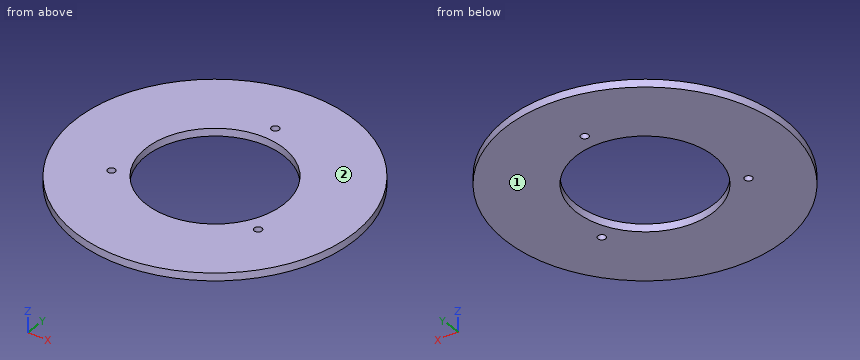
```python
from build123d import *

# Parameters (mm, degrees)
SKETCH1_R           = 91
SKETCH1_R_2         = 45
SKETCH1_R_3         = 2.5
BOSS_EXTRUDE1_DEPTH = 5


with BuildPart() as part:
    # Sketch1 → Boss-Extrude1 (new body)
    with BuildSketch(Plane.XY):
        Circle(SKETCH1_R)
        Circle(SKETCH1_R_2, mode=Mode.SUBTRACT)
        with Locations((0, 55)):
            Circle(SKETCH1_R_3, mode=Mode.SUBTRACT)
        with Locations((47.631397208, -27.5)):
            Circle(SKETCH1_R_3, mode=Mode.SUBTRACT)
        with Locations((-47.631397208, -27.5)):
            Circle(SKETCH1_R_3, mode=Mode.SUBTRACT)
    extrude(amount=BOSS_EXTRUDE1_DEPTH)


solid = part.part
```
For this review, take the finished solid that the model builds, in its own axes (mm). Face numbers are marked on the shaded views. Coordinates: 2 decimals unless noted, no trailing zeros. Loops run counter-clockwise (first coordinate to the right, second up) from the corner with the lowest first, then second, coordinate; pieces in that order, holes last. Notation, with made-up numbers: (73, 85.25) - (85, 85.25) arc R20 ccw to (85, 112.25) - close; hole circle Ø5 at (76, 28.25). An arc over 180 degrees is marked (long way). Use one line per item in the form item = value. Start each with the question number.
1) To check wall thickness, follow probe 1 along Y at (x, z) = (0, 1.85); probe 2 along X at (y, z) = (9, 0.35); probe 3 along X at (y, z) = (36, 3.05). State the ranges of each line that lie inside material, in increasing order. Write a range as from..to.
2) Take a section at D-D (y = -27.5). State the section outline as (x, z) points, plus the area to 3 significant figures.
3) Take a section at A-A (x = 0). State the section outline as (y, z) points.
4) Take a section at C-C (z = 2.8). State the section outline as (x, y) points.
5) For pin 1 (1 mm diameter, centred on x = -13, z = 2, fed in from -Y); pin 2 (3 mm diameter, centred on x = 0, y = 55, fed in from -Z); pin 3 (1 mm diameter, centred on y = 58.5, z = 0.5, fed in from -X); pin 4 (1.5 mm diameter, centred on x = -37, z = 2, fed in from +Y), all flat-tipped, find the tip position at first contact; note any pin that passes through.
6) Take a section at B-B (y = 0). State the section outline as (x, z) points.
7) Draft analysis for pull direction Z (two halves, no side actions). For the marked faces 1 and 2, state which applies: released by +Z, released by -Z, zero draft, split by the parting line, or undercut.
From the geometry:
q1.probe_1 = -91..-45, 45..52.5, 57.5..91
q1.probe_2 = -90.55..-44.09, 44.09..90.55
q1.probe_3 = -83.58..-27, 27..83.58
q2.outline = (-86.75, 0) - (-50.13, 0) - (-50.13, 5) - (-86.75, 5) - close; (-45.13, 0) - (-35.62, 0) - (-35.62, 5) - (-45.13, 5) - close; (35.62, 0) - (45.13, 0) - (45.13, 5) - (35.62, 5) - close; (50.13, 0) - (86.75, 0) - (86.75, 5) - (50.13, 5) - close
q2.area = 461 mm2
q3.outline = (-91, 0) - (-45, 0) - (-45, 5) - (-91, 5) - close; (45, 0) - (52.5, 0) - (52.5, 5) - (45, 5) - close; (57.5, 0) - (91, 0) - (91, 5) - (57.5, 5) - close
q4.outline = circle Ø182 at (0, 0); hole circle Ø5 at (-47.63, -27.5); hole circle Ø90 at (0, 0); hole circle Ø5 at (0, 55); hole circle Ø5 at (47.63, -27.5)
q5.pin_1 = -90.14
q5.pin_2 = through
q5.pin_3 = -70.12
q5.pin_4 = 83.47
q6.outline = (-91, 0) - (-45, 0) - (-45, 5) - (-91, 5) - close; (45, 0) - (91, 0) - (91, 5) - (45, 5) - close
q7.face_1 = released by -Z
q7.face_2 = released by +Z
